from build123d import *

# Parameters (mm, degrees)
EXTRUDE_1_DEPTH = 16
CHAMFER_1_SIZE  = 12


with BuildPart() as part:
    # 草图1 → 凸台-拉伸1 (new body)
    with BuildSketch(Plane.XY):
        Polygon((-599, -819), (-375, -819), (-375, -899), (375, -899), (375, -819), (599, -819), (599, 500), (-599, 500), align=None)
    extrude(amount=EXTRUDE_1_DEPTH)

    # 倒角1
    chamfer_1_edges = [part.edges().sort_by_distance(p)[0] for p in [
        (-599, 500, 8),
        (599, 500, 8),
    ]]
    chamfer(chamfer_1_edges, length=CHAMFER_1_SIZE)


solid = part.part
The listing builds one solid part. Answer for the finished solid, in the listing's coordinates (mm). Give positions to 0.01 mm unless a question says otherwise; leave off trailing zeros. Loops run counter-clockwise (first coordinate to the right, second up) from the corner with the lowest first, then second, coordinate; pieces in that order, holes last. Notation, with made-up numbers: (8.25, -11) - (53.25, -11) arc R25 ccw to (53.25, 11) - close; hole circle Ø3 at (-33, 89). An arc over 180 degrees is marked (long way). Write each question's results on one line, items separated by ' | '.
1. Find section A-A, the plane z = 12. Write down the section's boundary in (x, y).
Resolved:
outline: (-599, -819) - (-375, -819) - (-375, -899) - (375, -899) - (375, -819) - (599, -819) - (599, 488) - (587, 500) - (-587, 500) - (-599, 488) - close
2. A flat-ended cylindrical pin translates along its axis: P1, Ø8, axis at y = -878, z = 10.5, coming from the -X side. Find the tip coordinate at first contact, or state that the pin passes through.
Resolved:
P1: stops at x = -375
3. Find section B-B, the plane x = -445. Write down the section's boundary in (y, z), then the cut area to 3 significant figures.
Resolved:
outline: (-819, 0) - (500, 0) - (500, 16) - (-819, 16) - close | area: 21,100 mm^2
4. Consider probe 1 along Y at (x, z) = (440, 3.25). Determine where the line is inside the solid, lowest interval first. Write a range as from..to.
Resolved:
probe 1: y = -819..500
